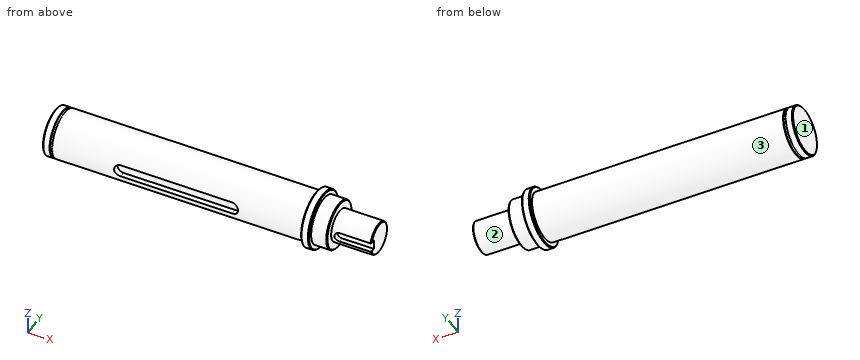
from build123d import *

# Parameters (mm, degrees)
CHAMFER_1_SIZE      = 0.5
CUT_EXTRUDE_1_DEPTH = 4
CUT_EXTRUDE_2_DEPTH = 3.5


with BuildPart() as part:
    # 草图1 → 旋转1 (revolve)
    with BuildSketch(Plane.XY, mode=Mode.PRIVATE) as revolve_1_sk:
        Polygon((0, 0), (0, 15), (4.4, 15), (4.4, 14.3), (6, 14.3), (6, 15), (164, 15), (164, 18), (169, 18), (169, 15), (179, 15), (179, 10), (204, 10), (204, 0), align=None)
    revolve(revolve_1_sk.sketch.rotate(Axis((0, 0, 0), (1, 0, 0)), 90), axis=Axis((0, 0, 0), (1, 0, 0)))

    # 倒角1
    chamfer_1_edges = [part.edges().sort_by_distance(p)[0] for p in [
        (204, 0, -10),
        (179, 0, -15),
        (169, 0, -18),
        (164, 0, -18),
        (0, 0, -15),
    ]]
    chamfer(chamfer_1_edges, length=CHAMFER_1_SIZE)

    # 草图2 → 切除-拉伸1 (cut)
    with BuildSketch(Plane(origin=(0, -15, 0), x_dir=(-1, 0, 0), z_dir=(0, -1, 0))):
        with BuildLine():
            Line((-49, -4), (-119, -4))
            ThreePointArc((-119, -4), (-123, 0), (-119, 4))
            Line((-119, 4), (-49, 4))
            ThreePointArc((-49, 4), (-45, 0), (-49, -4))
        make_face()
    extrude(amount=-CUT_EXTRUDE_1_DEPTH, mode=Mode.SUBTRACT)

    # 草图3 → 切除-拉伸2 (cut)
    with BuildSketch(Plane(origin=(0, -10, 0), x_dir=(-1, 0, 0), z_dir=(0, -1, 0))):
        with BuildLine():
            Line((-204, 3), (-184, 3))
            ThreePointArc((-184, 3), (-181, 0), (-184, -3))
            Line((-184, -3), (-204, -3))
            ThreePointArc((-204, -3), (-207, 0), (-204, 3))
        make_face()
    extrude(amount=-CUT_EXTRUDE_2_DEPTH, mode=Mode.SUBTRACT)


solid = part.part
Part model, mm, in its own coordinate system. Face numbers are marked on the shaded views. A direction names the side the tool comes from. Round coordinates to 2 decimals unless told otherwise and drop trailing zeros. Loops run counter-clockwise (first coordinate to the right, second up) from the corner with the lowest first, then second, coordinate; pieces in that order, holes last. Notation, with made-up numbers: (8.5, -11.75) - (48.5, -11.75) arc R12 ccw to (48.5, -6.75) - close; hole circle Ø1 at (80.5, 83). An arc over 180 degrees is marked (long way). Answer as a JSON object with one key per item and string values.
Item 1: Pin check, flat tips, straight feed: pin 1 (1.5 mm diameter, centred on x = 117.5, z = 14, fed in from +Y); pin 2 (3.5 mm diameter, centred on x = 197, y = -8.5, fed in from -Z); pin 3 (2 mm diameter, centred on y = 9, z = -13.5, fed in from +X). Stop position of each tip, or through.
Output:
{"pin 1": "y = 7.03", "pin 2": "z = -7.38", "pin 3": "x = 169"}
Item 2: Wall check: L1, parallel to Z at x = 96, y = -0.5; L2, parallel to X at y = -7, z = 0.5; L3, parallel to X at y = 5, z = 15. Give the ranges that are in metal, low to high.
Output:
{"L1": "-14.99 to 14.99", "L2": "0 to 181.04", "L3": "164 to 169"}
Item 3: Band-saw the part on B-B on x = 34. List the corners of the cut face in (y, z).
Output:
{"outline": "circle Ø30 at (0, 0)"}
Item 4: Band-saw the part on C-C on x = 62. List the corners of the cut face in (y, z), plus the area to 3 significant figures.
Output:
{"outline": "(-14.46, -4) arc R15 ccw (long way) to (-14.46, 4) - (-11, 4) - (-11, -4) - close", "area": "676 mm2"}
Item 5: Tool access for the marked faces 1, 2 and 3: list every direction of +Z, -Z, +X, -X, +Y, -Y with a clear straight run to the whole face (end or side of a thin tool).
Output:
{"face 1": "+Z, -Z, -X, +Y, -Y", "face 2": "+X", "face 3": "-X"}
